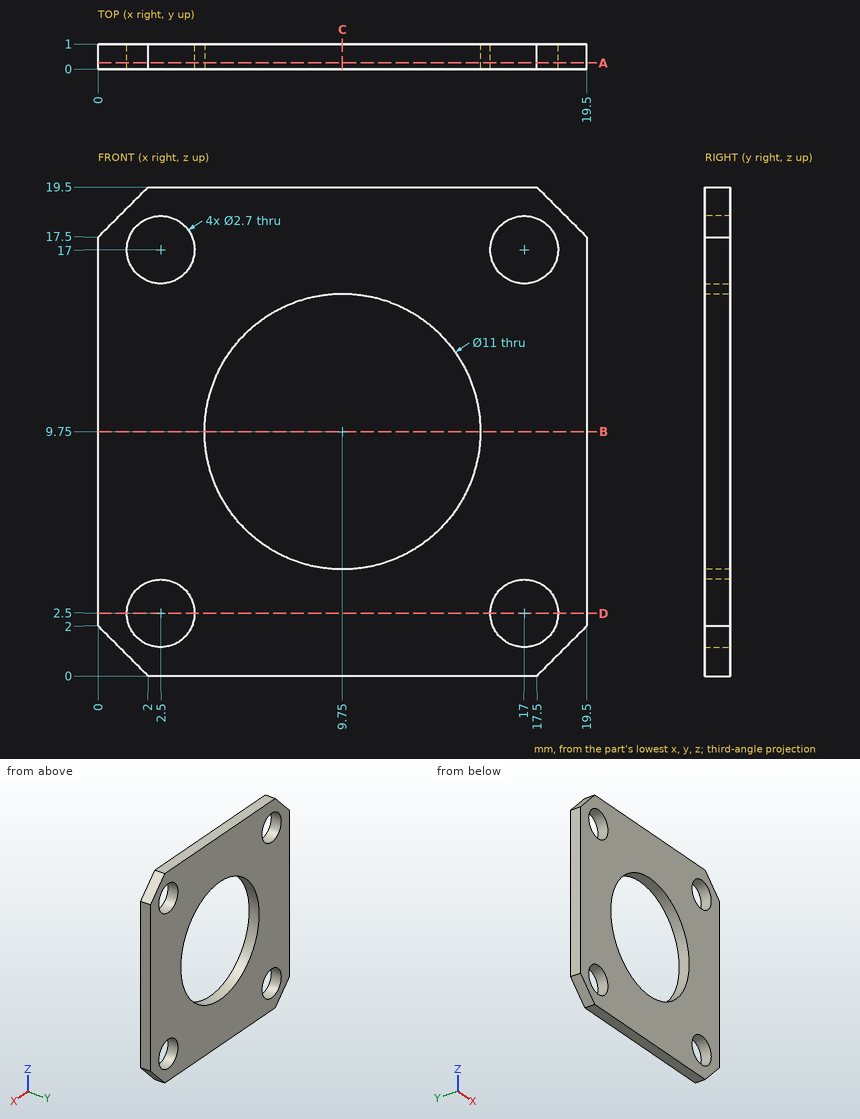
Geometry check sheet. Reference: drawing and pictorial views, mm from the part's lowest x, y, z. Give positions to 0.01 mm unless a question says otherwise; leave off trailing zeros. Order: outer loops, then holes, each group sorted by start corner. A loop starts at its lowest first (then second) coordinate and runs counter-clockwise, first axis right, second up. Notation, with made-up numbers: M 38.25,35 L 54.25,35 A13 cw 54.25,45 Z; hole C 13.25,77 d8. An arc over 180 degrees is marked long. Use one line per item in the form item = value. Start each with the question number.
Q1. Section check D-D (z = 2.5). Enter the section's corners in (x, y).
Q2. Section check C-C (x = 9.75). Enter the section's corners in (y, z), then the cut area to 3 significant figures.
Q3. Go/stop test with flat-tipped pins: pin 1 Ø10 at (x, z) = (7, 13) entering from -Y; pin 2 Ø6.5 at (x, z) = (9.75, 9.75) entering from -Y. Record where each tip stops, or that it passes through.
Q4. Scan lines: line 1 along X through (y, z) = (0.8, 17); line 2 along Z through (x, y) = (3.5, 0.55); line 3 along Z through (x, y) = (16.25, 0.4). Record each from-to range of solid material in increasing order. Write a range as [from, to].
Q5. Section check A-A (y = 0.25). Enter the section's corners in (x, z).
Q6. Section check B-B (z = 9.75). Enter the section's corners in (x, y).
Evaluation:
q1.outline = M 0,0 L 1.15,0 L 1.15,1 L 0,1 Z; M 3.85,0 L 15.65,0 L 15.65,1 L 3.85,1 Z; M 18.35,0 L 19.5,0 L 19.5,1 L 18.35,1 Z
q2.outline = M 0,0 L 1,0 L 1,4.25 L 0,4.25 Z; M 0,15.25 L 1,15.25 L 1,19.5 L 0,19.5 Z
q2.area = 8.50 mm2
q3.pin_1 = 0
q3.pin_2 = through
q4.line_1 = [0, 1.15], [3.85, 15.65], [18.35, 19.5]
q4.line_2 = [0, 1.59], [3.41, 16.09], [17.91, 19.5]
q4.line_3 = [0, 1.38], [3.62, 15.88], [18.12, 19.5]
q5.outline = M 0,2 L 2,0 L 17.5,0 L 19.5,2 L 19.5,17.5 L 17.5,19.5 L 2,19.5 L 0,17.5 Z; hole C 2.5,2.5 d2.7; hole C 2.5,17 d2.7; hole C 9.75,9.75 d11; hole C 17,2.5 d2.7; hole C 17,17 d2.7
q6.outline = M 0,0 L 4.25,0 L 4.25,1 L 0,1 Z; M 15.25,0 L 19.5,0 L 19.5,1 L 15.25,1 Z
